```python
from build123d import *

# Parameters (mm, degrees)
SKETCH_1_W                = 128
SKETCH_1_H                = 80
EXTRUDE_1_DEPTH           = 12
HOLE_WIZARD_1_D           = 9
HOLE_WIZARD_1_CBORE_D     = 15
HOLE_WIZARD_1_CBORE_DEPTH = 9
HOLE_WIZARD_9_0_9_1_D     = 9
CHAMFER_1_SIZE            = 5


with BuildPart() as part:
    # 草图1 → 凸台-拉伸1 (new body)
    with BuildSketch(Plane(origin=(0, 0, 0), x_dir=(0, 0, -1), z_dir=(1, 0, 0))):
        Rectangle(SKETCH_1_W, SKETCH_1_H)
    extrude(amount=EXTRUDE_1_DEPTH)

    # 打孔尺寸(%根据)内六角圆柱头螺钉的类型1 (through all)
    with Locations(Plane.ZY):
        with Locations((-37, 27.5), (-37, -27.5), (37, 27.5), (37, -27.5)):
            CounterBoreHole(HOLE_WIZARD_1_D / 2, HOLE_WIZARD_1_CBORE_D / 2, HOLE_WIZARD_1_CBORE_DEPTH)

    # Ø9.0 (9) 直径孔1 (through all)
    with Locations(Plane(origin=(12, 0, 0), x_dir=(0, 0, -1), z_dir=(1, 0, 0))):
        with Locations((-55, -5), (55, -5)):
            Hole(HOLE_WIZARD_9_0_9_1_D / 2)

    # 倒角1
    chamfer_1_edges = [part.edges().sort_by_distance(p)[0] for p in [
        (6, -40, -64),
        (6, -40, 64),
        (6, 40, 64),
        (6, 40, -64),
    ]]
    chamfer(chamfer_1_edges, length=CHAMFER_1_SIZE)


solid = part.part
```
Could you check a few things on this model? Use its own coordinates, in mm. A direction names the side the tool comes from. Round coordinates to 2 decimals unless told otherwise and drop trailing zeros. Loops run counter-clockwise (first coordinate to the right, second up) from the corner with the lowest first, then second, coordinate; pieces in that order, holes last. Notation, with made-up numbers: (16, 84) -> (43, 84) arc R17 cw to (43, 105) -> close; hole circle Ø3 at (-16.75, 9.25). An arc over 180 degrees is marked (long way). Put each result on its own line as item: value.
Q1. I want a section at A-A on z = -55. Write out the boundary of the cut face in (x, y).
Checks:
outline: (0, -40) -> (12, -40) -> (12, -9.5) -> (0, -9.5) -> close; (0, -0.5) -> (12, -0.5) -> (12, 40) -> (0, 40) -> close
Q2. Please list where these lines run through material, in increasing order: line 1 (Y direction, x = 4.75, z = -37); line 2 (Z direction, x = 3, y = -24.5); line 3 (Y direction, x = 5.75, z = -42). Write a range as from..to.
Checks:
line 1: -40..-35, -20..20, 35..40
line 2: -64..-43.87, -30.13..30.13, 43.87..64
line 3: -40..-33.09, -21.91..21.91, 33.09..40
Q3. I want a section at D-D on z = -37. Write out the boundary of the cut face in (x, y), and give its area (3 significant figures).
Checks:
outline: (0, -40) -> (12, -40) -> (12, -32) -> (9, -32) -> (9, -35) -> (0, -35) -> close; (0, -20) -> (9, -20) -> (9, -23) -> (12, -23) -> (12, 23) -> (9, 23) -> (9, 20) -> (0, 20) -> close; (0, 35) -> (9, 35) -> (9, 32) -> (12, 32) -> (12, 40) -> (0, 40) -> close
area: 636 mm2
Q4. Which directions (+Z, -Z, +X, -X, +Y, -Y) give clear straight access to the entire face, cutting with the end or side of a thin tool? Please do faces 5 (the flat face through (9, -27, 42)), 6 (the flat face through (6, 0, -64)).
Checks:
face 5: -X
face 6: -Z, +X, -X, +Y, -Y
Q5. For pin 1 Ø12 at (y, z) = (-27.5, -37) entering from -X; pin 2 Ø17 at (y, z) = (27.5, -37) entering from +X, each with a flat end and sliding along its axis, tell me the tip position at first contact or that it passes through.
Checks:
pin 1: x = 9
pin 2: x = 12
Q6. Thinking about a two-plate mould opening in Y: for faces 1 (the flat face through (6, 40, 1)), 2 (the cylindrical face through (4.437, 27.83, -44.493)), 3 (the flat face through (6, -38, 61)), 4 (the cylindrical face through (5.916, -3.648, -50.708)), which applies, pulls with the +Y half, pulls with the -Y half, needs draft (parallel to the pull), parting line crosses it, or undercut?
Checks:
face 1: pulls with the +Y half
face 2: undercut
face 3: pulls with the -Y half
face 4: undercut
Q7. I want a section at B-B on x = 2.5. Write out the boundary of the cut face in (y, z).
Checks:
outline: (-40, -59) -> (-35, -64) -> (35, -64) -> (40, -59) -> (40, 59) -> (35, 64) -> (-35, 64) -> (-40, 59) -> close; hole circle Ø15 at (-27.5, -37); hole circle Ø15 at (-27.5, 37); hole circle Ø9 at (-5, -55); hole circle Ø9 at (-5, 55); hole circle Ø15 at (27.5, -37); hole circle Ø15 at (27.5, 37)
Q8. I want a section at C-C on y = -5. Write out the boundary of the cut face in (x, z).
Checks:
outline: (0, -64) -> (12, -64) -> (12, -59.5) -> (0, -59.5) -> close; (0, -50.5) -> (12, -50.5) -> (12, 50.5) -> (0, 50.5) -> close; (0, 59.5) -> (12, 59.5) -> (12, 64) -> (0, 64) -> close
